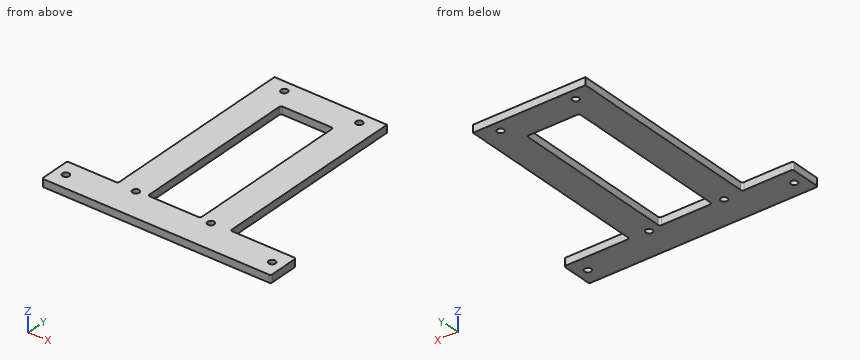
from build123d import *

# Parameters (mm, degrees)
SKETCH1_R           = 9
BOSS_EXTRUDE1_DEPTH = 20


with BuildPart() as part:
    # Sketch1 → Boss-Extrude1 (new body)
    with BuildSketch(Plane.XY):
        with BuildLine():
            Line((5, 0), (605, 0))
            ThreePointArc((605, 0), (608.535533906, 1.464466094), (610, 5))
            Line((610, 5), (610, 80))
            ThreePointArc((610, 80), (608.535533906, 83.535533906), (605, 85))
            Line((605, 85), (440, 85))
            ThreePointArc((440, 85), (436.464466094, 86.464466094), (435, 90))
            Line((435, 90), (435, 612.5))
            Line((435, 612.5), (135, 612.5))
            Line((135, 612.5), (135, 90))
            ThreePointArc((135, 90), (133.535533906, 86.464466094), (130, 85))
            Line((130, 85), (5, 85))
            ThreePointArc((5, 85), (1.464466094, 83.535533906), (0, 80))
            Line((0, 80), (0, 5))
            ThreePointArc((0, 5), (1.464466094, 1.464466094), (5, 0))
        make_face()
        with Locations((30, 42.5)):
            Circle(SKETCH1_R, mode=Mode.SUBTRACT)
        with Locations((580, 42.5)):
            Circle(SKETCH1_R, mode=Mode.SUBTRACT)
        with Locations((185, 582.5)):
            Circle(SKETCH1_R, mode=Mode.SUBTRACT)
        with Locations((385, 582.5)):
            Circle(SKETCH1_R, mode=Mode.SUBTRACT)
        with Locations((185, 82.5)):
            Circle(SKETCH1_R, mode=Mode.SUBTRACT)
        with Locations((385, 82.5)):
            Circle(SKETCH1_R, mode=Mode.SUBTRACT)
        with BuildLine():
            Line((220, 85), (350, 85))
            ThreePointArc((350, 85), (353.535533906, 86.464466094), (355, 90))
            Line((355, 90), (355, 527.5))
            ThreePointArc((355, 527.5), (353.535533906, 531.035533906), (350, 532.5))
            Line((350, 532.5), (220, 532.5))
            ThreePointArc((220, 532.5), (216.464466094, 531.035533906), (215, 527.5))
            Line((215, 527.5), (215, 90))
            ThreePointArc((215, 90), (216.464466094, 86.464466094), (220, 85))
        make_face(mode=Mode.SUBTRACT)
    extrude(amount=BOSS_EXTRUDE1_DEPTH)


solid = part.part
Design review of the part built by this model. Coordinates are the model's own, in mm. Coordinates: 2 decimals unless noted, no trailing zeros. Order: outer loops, then holes, each group sorted by start corner. A loop starts at its lowest first (then second) coordinate and runs counter-clockwise, first axis right, second up. Notation, with made-up numbers: (-16, -27.75) - (-6, -27.75) arc R18 ccw to (-6, -17.75) - close; hole circle Ø2 at (-38.5, 52). An arc over 180 degrees is marked (long way). Put each result on its own line as item: value.
1) Take a section at D-D, the plane z = 16.25. Give the boundary of the cut face in (x, y).
Response values:
outline: (0, 5) arc R5 ccw to (5, 0) - (605, 0) arc R5 ccw to (610, 5) - (610, 80) arc R5 ccw to (605, 85) - (440, 85) arc R5 cw to (435, 90) - (435, 612.5) - (135, 612.5) - (135, 90) arc R5 cw to (130, 85) - (5, 85) arc R5 ccw to (0, 80) - close; hole circle Ø18 at (30, 42.5); hole circle Ø18 at (185, 82.5); hole circle Ø18 at (185, 582.5); hole (215, 90) arc R5 ccw to (220, 85) - (350, 85) arc R5 ccw to (355, 90) - (355, 527.5) arc R5 ccw to (350, 532.5) - (220, 532.5) arc R5 ccw to (215, 527.5) - close; hole circle Ø18 at (385, 82.5); hole circle Ø18 at (385, 582.5); hole circle Ø18 at (580, 42.5)
2) Insertion check: P1, Ø20.5, axis at x = 185, y = 82.5, coming from the -Z side; P2, Ø10, axis at y = 400, z = 11, coming from the -X side; P3, Ø11, axis at x = 385, y = 82.5, coming from the -Z side; P4, Ø8, axis at y = 329.5, z = 8, coming from the +X side. Each pin has a flat end and moves straight along its axis. Give the tip position at first contact, or say it passes through.
Response values:
P1: stops at z = 0
P2: stops at x = 135
P3: passes through
P4: stops at x = 435
3) Take a section at A-A, the plane x = 228. Give the boundary of the cut face in (y, z), and give its area (3 significant figures).
Response values:
outline: (0, 0) - (85, 0) - (85, 20) - (0, 20) - close; (532.5, 0) - (612.5, 0) - (612.5, 20) - (532.5, 20) - close
area: 3,300 mm²
4) Take a section at B-B, the plane y = 42.5. Give the boundary of the cut face in (x, z).
Response values:
outline: (0, 0) - (21, 0) - (21, 20) - (0, 20) - close; (39, 0) - (571, 0) - (571, 20) - (39, 20) - close; (589, 0) - (610, 0) - (610, 20) - (589, 20) - close
5) Wall thickness on L1, parallel to Y at x = 185, z = 13.25; L2, parallel to X at y = 81, z = 5.25; L3, parallel to X at y = 129, z = 4.5: over which ranges is each line inside the solid? List them lowest first. Write a range as from..to.
Response values:
L1: y = 0..73.5, 91.5..573.5, 591.5..612.5
L2: x = 0.1..176.13, 193.87..376.13, 393.87..609.9
L3: x = 135..215, 355..435
6) Take a section at C-C, the plane y = 462. Give the boundary of the cut face in (x, z), and give its area (3 significant figures).
Response values:
outline: (135, 0) - (215, 0) - (215, 20) - (135, 20) - close; (355, 0) - (435, 0) - (435, 20) - (355, 20) - close
area: 3,200 mm²
